Verification items for the finished model (mm, model axes). Face numbers are marked on the shaded views. A direction names the side the tool comes from. Coordinates: 2 decimals unless noted, no trailing zeros. Loops run counter-clockwise (first coordinate to the right, second up) from the corner with the lowest first, then second, coordinate; pieces in that order, holes last. Notation, with made-up numbers: (61, -32.5) - (65, -32.5) arc R8 cw to (65, -23.5) - close; hole circle Ø8 at (52.5, 9). An arc over 180 degrees is marked (long way). One line per item, written item: value. Start each with the question number.
(1) Thickness scan on probe 1 along Y at (x, z) = (4, 4.4); probe 2 along X at (y, z) = (5.75, -5.25); probe 3 along Y at (x, z) = (3.5, -5.5). Record the ranges inside material, lowest first. Write a range as [from, to].
(2) Gauge pin test, flat ends, axial feed: P1, Ø3, axis at x = 3, z = 3.5, coming from the +Y side; P2, Ø2, axis at x = -4, y = 8.25, coming from the -Z side; P3, Ø2.5, axis at x = -3, z = -1.5, coming from the +Y side; P4, Ø5, axis at y = 15, z = 1.5, coming from the -X side. Record the tip position at first contact, or that the pin passes through.
(3) Section check B-B (y = 7.25). Record the boundary of the cut face in (x, z), plus the area to 3 significant figures.
(4) Section check A-A (x = 0). Record the boundary of the cut face in (y, z), plus the area to 3 significant figures.
(5) Section check C-C (z = -1.25). Record the boundary of the cut face in (x, y), plus the area to 3 significant figures.
(6) Section check D-D (y = 3). Record the boundary of the cut face in (x, z), plus the area to 3 significant figures.
(7) Draft check along Y on the marked faces 1, 2, 3 and 4. Enter one of: +Y half, -Y half, draft (parallel to the pull), parting line (faces both ways), or undercut.
(8) Set-up check for the marked faces 5 and 6: record each of +Z, -Z, +X, -X, +Y, -Y from which the full face is reachable in a straight line by a thin tool's end or side.
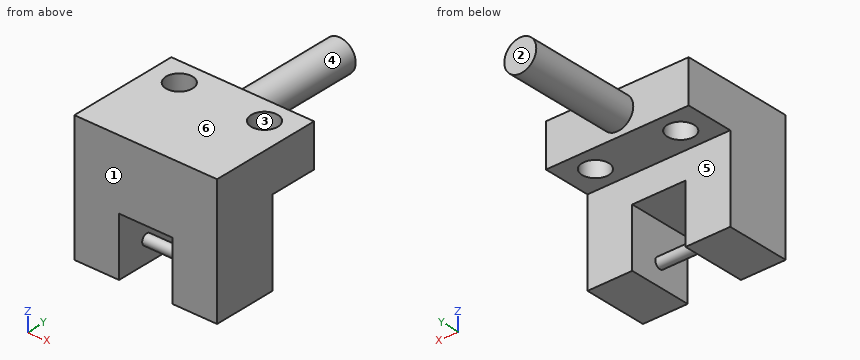
```python
from build123d import *

# Parameters (mm, degrees)
BOSS_EXTRUDE1_DEPTH = 6
SKETCH2_W           = 13.4
SKETCH2_H           = 4
BOSS_EXTRUDE2_DEPTH = 4.5
SKETCH3_R           = 1.5
BOSS_EXTRUDE3_DEPTH = 10.5
SKETCH4_R           = 1.25
CUT_EXTRUDE1_DEPTH  = 10.5
SKETCH5_R           = 0.5
BOSS_EXTRUDE4_DEPTH = 5


with BuildPart() as part:
    # Sketch1 → Boss-Extrude1 (new body)
    with BuildSketch(Plane(origin=(0, 0, 0), x_dir=(1, 0, 0), z_dir=(0, 1, 0))):
        Polygon((2.5, 6), (6.7, 6), (6.7, -6), (-6.7, -6), (-6.7, 6), (-2.5, 6), (-2.5, 0.5), (2.5, 0.5), align=None)
    extrude(amount=BOSS_EXTRUDE1_DEPTH)

    # Sketch2 → Boss-Extrude2 (add)
    with BuildSketch(Plane(origin=(0, 6, 0), x_dir=(1, 0, 0), z_dir=(0, 1, 0))):
        with Locations((0, -4)):
            Rectangle(SKETCH2_W, SKETCH2_H)
    extrude(amount=BOSS_EXTRUDE2_DEPTH)

    # Sketch3 → Boss-Extrude3 (add)
    with BuildSketch(Plane(origin=(0, 10.5, 0), x_dir=(1, 0, 0), z_dir=(0, 1, 0))):
        with Locations(Location((0, -4, 0), (0, 0, 90))):
            Circle(SKETCH3_R)
    extrude(amount=BOSS_EXTRUDE3_DEPTH)

    # Sketch4 → Cut-Extrude1 (cut)
    with BuildSketch(Plane(origin=(0, 0, 2), x_dir=(-1, 0, 0), z_dir=(0, 0, -1))):
        with Locations((-4, 8.25)):
            Circle(SKETCH4_R)
        with Locations((4, 8.25)):
            Circle(SKETCH4_R)
    extrude(amount=-CUT_EXTRUDE1_DEPTH, mode=Mode.SUBTRACT)

    # Sketch5 → Boss-Extrude4 (add)
    with BuildSketch(Plane.ZY.offset(-2.5)):
        with Locations(Location((-4, 3, 0), (0, 0, 180))):
            Circle(SKETCH5_R)
    extrude(amount=BOSS_EXTRUDE4_DEPTH)


solid = part.part
```
Responses:
1. probe 1: y = [0, 7], [9.5, 10.5]
1. probe 2: x = [-6.7, -2.5], [2.5, 6.7]
1. probe 3: y = [0, 6]
2. P1: stops at y = 10.5
2. P2: passes through
2. P3: stops at y = 6
2. P4: stops at x = -1.5
3. outline: (-6.7, 2) - (-4.75, 2) - (-4.75, 6) - (-6.7, 6) - close; (-3.25, 2) - (3.25, 2) - (3.25, 6) - (-3.25, 6) - close; (4.75, 2) - (6.7, 2) - (6.7, 6) - (4.75, 6) - close
3. area: 41.6 mm²
4. outline: (0, -0.5) - (6, -0.5) - (6, 2) - (10.5, 2) - (10.5, 2.5) - (21, 2.5) - (21, 5.5) - (10.5, 5.5) - (10.5, 6) - (0, 6) - close; circle Ø1 at (3, -4)
4. area: 89.3 mm²
5. outline: (-6.7, 0) - (-2.5, 0) - (-2.5, 6) - (-6.7, 6) - close; (2.5, 0) - (6.7, 0) - (6.7, 6) - (2.5, 6) - close
5. area: 50.4 mm²
6. outline: (-6.7, -6) - (-2.5, -6) - (-2.5, -4.5) - (2.5, -4.5) - (2.5, -6) - (6.7, -6) - (6.7, 6) - (-6.7, 6) - close; hole (-2.5, -3.5) - (2.5, -3.5) - (2.5, -0.5) - (-2.5, -0.5) - close
6. area: 138 mm²
7. face 1: -Y half
7. face 2: +Y half
7. face 3: undercut
7. face 4: draft
8. face 5: -Z, +X, -X, +Y
8. face 6: +Z, +X, -X, +Y, -Y
